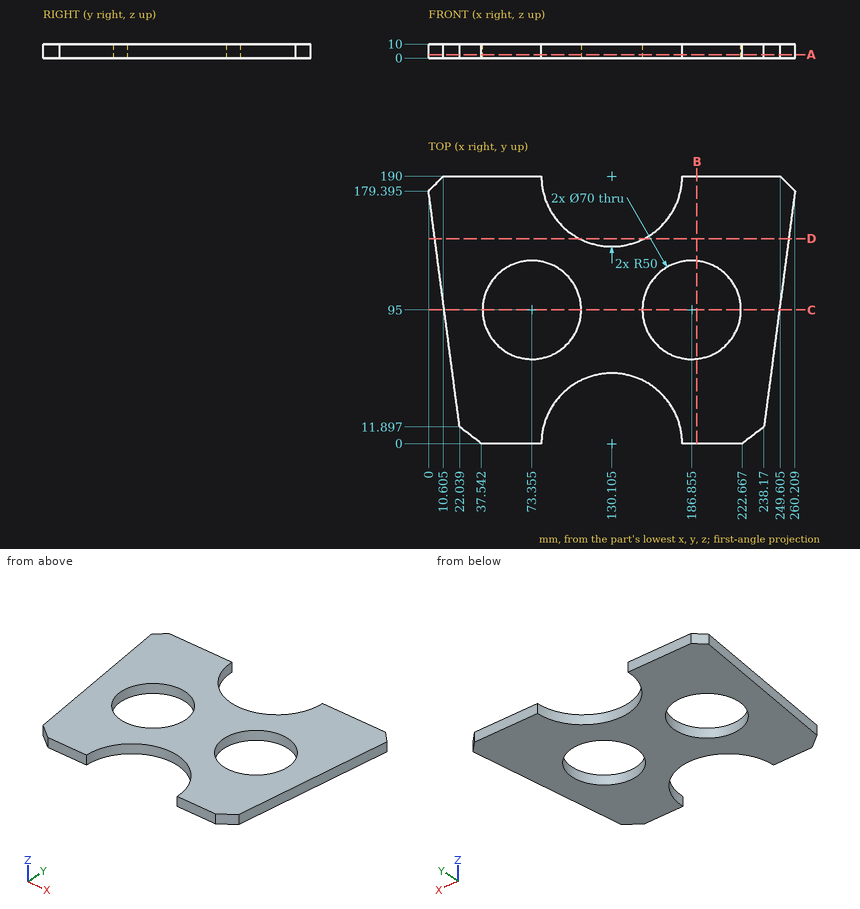
Geometry check sheet. Reference: drawing and pictorial views, mm from the part's lowest x, y, z. Give positions to 0.01 mm unless a question says otherwise; leave off trailing zeros. Order: outer loops, then holes, each group sorted by start corner. A loop starts at its lowest first (then second) coordinate and runs counter-clockwise, first axis right, second up. Notation, with made-up numbers: M -25,7 L -18,7 A30 ccw -18,29 Z; hole C 17.5,5 d9. An arc over 180 degrees is marked long. Use one line per item in the form item = value. Start each with the question number.
Q1. Section check B-B (x = 190.5). Enter the section's corners in (y, z).
Q2. Section check D-D (y = 145.5). Enter the section's corners in (x, z), then the cut area to 3 significant figures.
Q3. Scan lines: line 1 along X through (y, z) = (109, 5) (1 decimal); line 2 along X through (y, z) = (116, 1.5) (1 decimal); line 3 along Y through (x, z) = (155, 9.25) (1 decimal). Record each from-to range of solid material in increasing order. Write a range as [from, to].
Q4. Section check A-A (z = 2.5). Enter the section's corners in (x, y) (1 decimal), then the cut area to 3 significant figures.
Q5. Go/stop test with flat-tipped pins: pin 1 Ø1 at (y, z) = (155.5, 3) entering from -X; pin 2 Ø1 at (y, z) = (21, 2) entering from +X; pin 3 Ø4 at (y, z) = (98.5, 5.5) entering from -X; pin 4 Ø2 at (x, y) = (159.5, 112.5) entering from +Z. Record where each tip stops, or that it passes through.
Q6. Section check C-C (y = 95). Enter the section's corners in (x, z) (1 decimal).
Evaluation:
q1.outline = M 0,0 L 60.19,0 L 60.19,10 L 0,10 Z; M 129.81,0 L 190,0 L 190,10 L 129.81,10 Z
q2.outline = M 4.46,0 L 107.31,0 L 107.31,10 L 4.46,10 Z; M 152.9,0 L 255.75,0 L 255.75,10 L 152.9,10 Z
q2.area = 2,060 mm2
q3.line_1 = [9.3, 41.3], [105.4, 154.8], [218.9, 250.9]
q3.line_2 = [8.3, 45.4], [101.4, 158.9], [214.9, 251.9]
q3.line_3 = [43.4, 80.5], [109.5, 146.6]
q4.outline = M 0,179.4 L 22,11.9 L 37.5,0 L 80.1,0 A50 cw 180.1,0 L 222.7,0 L 238.2,11.9 L 260.2,179.4 L 249.6,190 L 180.1,190 A50 cw 80.1,190 L 10.6,190 Z; hole C 73.4,95 d70; hole C 186.9,95 d70
q4.area = 29,400 mm2
q5.pin_1 = 3.08
q5.pin_2 = 239.43
q5.pin_3 = 10.38
q5.pin_4 = through
q6.outline = M 11.1,0 L 38.4,0 L 38.4,10 L 11.1,10 Z; M 108.4,0 L 151.9,0 L 151.9,10 L 108.4,10 Z; M 221.9,0 L 249.1,0 L 249.1,10 L 221.9,10 Z
